Verification items for the finished model (mm, model axes). Face numbers are marked on the shaded views. A direction names the side the tool comes from. Give positions to 0.01 mm unless a question says otherwise; leave off trailing zeros. Loops run counter-clockwise (first coordinate to the right, second up) from the corner with the lowest first, then second, coordinate; pieces in that order, holes last. Notation, with made-up numbers: M -6.75,31 L 25.25,31 A17 cw 25.25,56 Z; hole C 21,85 d9. An arc over 180 degrees is marked long. Use CSV: the item, a comma, the result in double quotes.
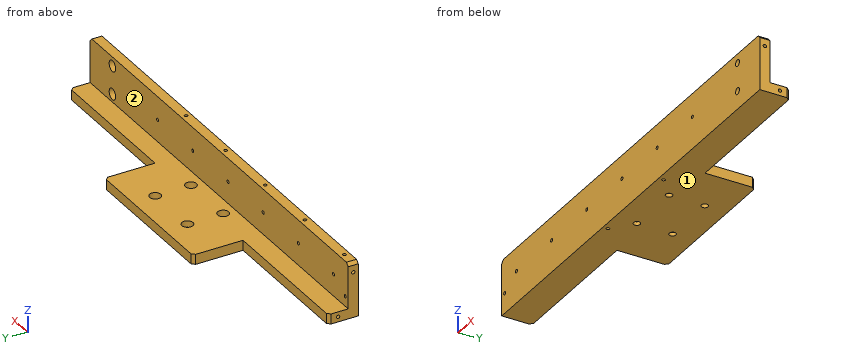
from build123d import *

# Parameters (mm, degrees)
SKETCH_2_W                   = 440
SKETCH_2_H                   = 80
EXTRUDE_1_DEPTH              = 10
SKETCH_3_W                   = 440
SKETCH_3_H                   = 10
EXTRUDE_2_DEPTH              = 45
SKETCH_5_W                   = 145
SKETCH_5_H                   = 50
CUT_EXTRUDE_2_DEPTH          = 239.379948821
HOLE_WIZARD_M6_1_D           = 6.6
HOLE_WIZARD_M6_1_DEPTH       = 22.25
HOLE_WIZARD_M6_1_CBORE_D     = 11
HOLE_WIZARD_M6_1_CBORE_DEPTH = 6.4
HOLE_WIZARD_M6_1_TIP         = 1.982840043
HOLE_WIZARD_M4_1_D           = 3.3
HOLE_WIZARD_M4_1_DEPTH       = 11.5
HOLE_WIZARD_M4_1_TIP         = 0.991420021
HOLE_WIZARD_M4_2_D           = 3.3
HOLE_WIZARD_M4_2_DEPTH       = 11.5
HOLE_WIZARD_M4_2_TIP         = 0.991420021
CHAMFER_1_SIZE               = 3
HOLE_WIZARD_M6_2_D           = 6.6
HOLE_WIZARD_M6_2_DEPTH       = 17
HOLE_WIZARD_M6_2_CBORE_D     = 11
HOLE_WIZARD_M6_2_CBORE_DEPTH = 6.4
HOLE_WIZARD_M6_2_TIP         = 1.982840043
HOLE_WIZARD_M4_3_D           = 3.3
HOLE_WIZARD_M4_3_DEPTH       = 11.5
HOLE_WIZARD_M4_3_TIP         = 0.991420021
HOLE_WIZARD_M4_4_AT_2_COUNT  = 2
HOLE_WIZARD_M4_4_AT_2_PITCH  = 42.720018727
HOLE_WIZARD_M4_5_D           = 3.3
HOLE_WIZARD_M4_5_DEPTH       = 11.5
HOLE_WIZARD_M4_5_TIP         = 0.991420021


with BuildPart() as part:
    # 草图2 → 凸台-拉伸1 (new body)
    with BuildSketch(Plane.XY):
        with Locations((0, -40)):
            Rectangle(SKETCH_2_W, SKETCH_2_H)
    extrude(amount=EXTRUDE_1_DEPTH)

    # 草图3 → 凸台-拉伸2 (add)
    with BuildSketch(Plane.XY.offset(10)):
        with Locations((0, -75)):
            Rectangle(SKETCH_3_W, SKETCH_3_H)
    extrude(amount=EXTRUDE_2_DEPTH)

    # 草图5 → 切除-拉伸2 (cut, through all)
    with BuildSketch(Plane.XY.offset(10)):
        with Locations((-147.5, -25)):
            Rectangle(SKETCH_5_W, SKETCH_5_H)
        with Locations((147.5, -25)):
            Rectangle(SKETCH_5_W, SKETCH_5_H)
    extrude(amount=-CUT_EXTRUDE_2_DEPTH, mode=Mode.SUBTRACT)

    # M6 六角凹头螺钉的柱形沉头孔1
    with Locations(Plane.XY.offset(10)):
        with Locations((-27.5, -22.520483068), (27.5, -22.520483068), (27.5, -58), (-27.396175046, -58)):
            CounterBoreHole(HOLE_WIZARD_M6_1_D / 2, HOLE_WIZARD_M6_1_CBORE_D / 2, HOLE_WIZARD_M6_1_CBORE_DEPTH, depth=HOLE_WIZARD_M6_1_DEPTH)
            with Locations((0, 0, -(HOLE_WIZARD_M6_1_DEPTH + HOLE_WIZARD_M6_1_TIP / 2))):  # 118° drill point
                Cone(0, HOLE_WIZARD_M6_1_D / 2, HOLE_WIZARD_M6_1_TIP, mode=Mode.SUBTRACT)

    # M4 螺纹孔1
    with Locations(Plane(origin=(0, -70, 0), x_dir=(1, 0, 0), z_dir=(0, 1, 0))):
        with Locations((-195, -31.742753413), (-135, -31.742753413), (-75, -31.742753413), (-15, -31.742753413), (45, -31.742753413), (105, -31.742753413)):
            Hole(HOLE_WIZARD_M4_1_D / 2, depth=HOLE_WIZARD_M4_1_DEPTH)
            with Locations((0, 0, -(HOLE_WIZARD_M4_1_DEPTH + HOLE_WIZARD_M4_1_TIP / 2))):  # 118° drill point
                Cone(0, HOLE_WIZARD_M4_1_D / 2, HOLE_WIZARD_M4_1_TIP, mode=Mode.SUBTRACT)

    # M4 螺纹孔2
    with Locations(Plane.XY.offset(55)):
        with Locations((-205, -75), (-137.5, -75), (-70, -75), (-2.5, -75), (65, -75)):
            Hole(HOLE_WIZARD_M4_2_D / 2, depth=HOLE_WIZARD_M4_2_DEPTH)
            with Locations((0, 0, -(HOLE_WIZARD_M4_2_DEPTH + HOLE_WIZARD_M4_2_TIP / 2))):  # 118° drill point
                Cone(0, HOLE_WIZARD_M4_2_D / 2, HOLE_WIZARD_M4_2_TIP, mode=Mode.SUBTRACT)

    # 倒角1
    chamfer_1_edges = [part.edges().sort_by_distance(p)[0] for p in [
        (-220, -75, 55),
        (220, -75, 55),
        (-220, -50, 5),
        (-75, 0, 5),
        (75, 0, 5),
        (220, -50, 5),
    ]]
    chamfer(chamfer_1_edges, length=CHAMFER_1_SIZE)

    # M6 六角凹头螺钉的柱形沉头孔2
    with Locations(Plane(origin=(0, -70, 0), x_dir=(1, 0, 0), z_dir=(0, 1, 0))):
        with Locations((182, -18), (182, -46)):
            CounterBoreHole(HOLE_WIZARD_M6_2_D / 2, HOLE_WIZARD_M6_2_CBORE_D / 2, HOLE_WIZARD_M6_2_CBORE_DEPTH, depth=HOLE_WIZARD_M6_2_DEPTH)
            with Locations((0, 0, -(HOLE_WIZARD_M6_2_DEPTH + HOLE_WIZARD_M6_2_TIP / 2))):  # 118° drill point
                Cone(0, HOLE_WIZARD_M6_2_D / 2, HOLE_WIZARD_M6_2_TIP, mode=Mode.SUBTRACT)

    # M4 螺纹孔3
    with Locations(Plane(origin=(0, -70, 0), x_dir=(1, 0, 0), z_dir=(0, 1, 0))):
        with Locations((-215, -20)):
            Hole(HOLE_WIZARD_M4_3_D / 2, depth=HOLE_WIZARD_M4_3_DEPTH)
            with Locations((0, 0, -(HOLE_WIZARD_M4_3_DEPTH + HOLE_WIZARD_M4_3_TIP / 2))):  # 118° drill point
                Cone(0, HOLE_WIZARD_M4_3_D / 2, HOLE_WIZARD_M4_3_TIP, mode=Mode.SUBTRACT)

    # 草图17 → M4 螺纹孔4 (revolve, cut)
    with BuildSketch(Plane(origin=(-220, -75, 45), x_dir=(0, 0, 1), z_dir=(0, 1, 0))):
        Polygon((0, 0), (0, 12.491420021), (1.65, 11.5), (1.65, 0), align=None)
    hole_wizard_m4_4 = revolve(axis=Axis((-226.35, -75, 45), (1, 0, 0)), mode=Mode.SUBTRACT)

    # M4 螺纹孔4 at 2: M4 螺纹孔4 ×2
    with Locations(*[Vector(0, 0.35112344158839187, -0.9363291775690445) * (i * HOLE_WIZARD_M4_4_AT_2_PITCH) for i in range(1, HOLE_WIZARD_M4_4_AT_2_COUNT)]):
        add(hole_wizard_m4_4, mode=Mode.SUBTRACT)

    # 镜向1: M4 螺纹孔4 across plane
    add(hole_wizard_m4_4.mirror(Plane(origin=(0, 0, 0), x_dir=(0, 0, 1), z_dir=(1, 0, 0))), mode=Mode.SUBTRACT)

    # 镜向1 copy 1 sketch → 镜向1 copy 1 (revolve, cut)
    with BuildSketch(Plane(origin=(220, -60, 5), x_dir=(0, 0, 1), z_dir=(0, 1, 0))):
        Polygon((0, 0), (0, -12.491420021), (1.65, -11.5), (1.65, 0), align=None)
    revolve(axis=Axis((226.35, -60, 5), (1, 0, 0)), mode=Mode.SUBTRACT)

    # M4 螺纹孔5
    with Locations(Plane(origin=(0, 0, 0), x_dir=(-1, 0, 0), z_dir=(0, 0, -1))):
        with Locations((-47.5, -75), (47.5, -75)):
            Hole(HOLE_WIZARD_M4_5_D / 2, depth=HOLE_WIZARD_M4_5_DEPTH)
            with Locations((0, 0, -(HOLE_WIZARD_M4_5_DEPTH + HOLE_WIZARD_M4_5_TIP / 2))):  # 118° drill point
                Cone(0, HOLE_WIZARD_M4_5_D / 2, HOLE_WIZARD_M4_5_TIP, mode=Mode.SUBTRACT)


solid = part.part
(1) Tool access check on the marked faces 1 and 2. Record the directions out of +Z, -Z, +X, -X, +Y, -Y that give a thin tool (end or side, any length) a straight path to the whole face; none if there is none.
Calculated:
face 1,"-Z, +X, -X, +Y, -Y"
face 2,"+Z, +X, -X, +Y"
(2) Section check A-A on x = 84. Record the cut outline in (y, z).
Calculated:
outline,"M -80,0 L -50,0 L -50,10 L -70,10 L -70,55 L -80,55 Z"
(3) Scan lines: L1, parallel to Z at x = 216.25, y = -60; L2, parallel to X at y = -75, z = 3; L3, parallel to Y at x = 48, z = 10.5. Record each from-to range of solid material in increasing order. Write a range as from..to.
Calculated:
L1,"z = 0..3.35, 6.65..10"
L2,"x = -220..-49.15, -45.85..45.85, 49.15..220"
L3,"y = -80..-76.57, -73.43..-70"
(4) Depth check by flat-ended pin: pin 1 Ø4 at (x, z) = (-140.5, 27) entering from +Y; pin 2 Ø2 at (y, z) = (-75, 45) entering from +X; pin 3 Ø5.5 at (x, y) = (27, -25) entering from +Z. Enter the tip coordinate at first touch or a pass-through.
Calculated:
pin 1,"stops at y = -70"
pin 2,"stops at x = 208.11"
pin 3,"stops at z = 3.6"
